For this review, use the dimensioned drawing (mm, ordinates from the lowest corner) and the shaded views. Round coordinates to 2 decimals unless told otherwise and drop trailing zeros. Order: outer loops, then holes, each group sorted by start corner. A loop starts at its lowest first (then second) coordinate and runs counter-clockwise, first axis right, second up. Notation, with made-up numbers: M 64.25,-18.5 L 89.25,-18.5 A24 cw 89.25,7.5 Z; hole C 27.25,50.5 d6. An arc over 180 degrees is marked long. Put each result on its own line as item: value.
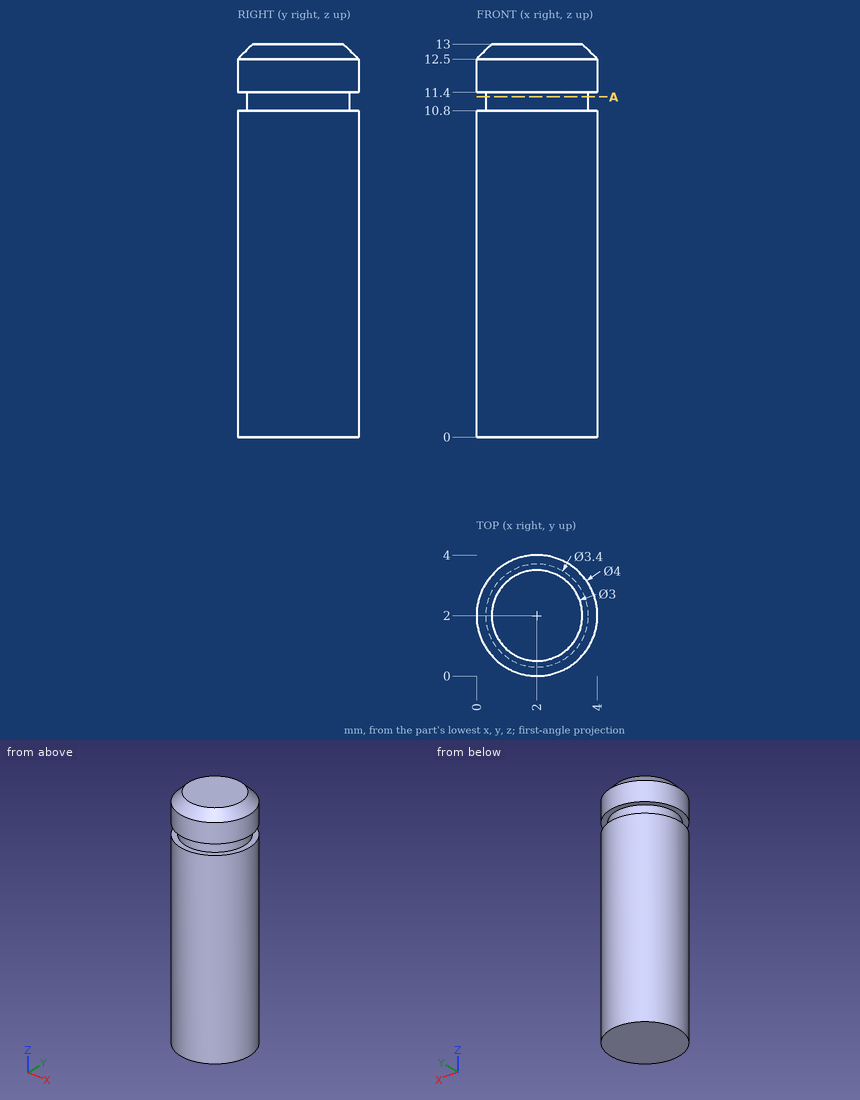
(1) To check wall thickness, follow L1, parallel to X at y = 3.05, z = 11.75; L2, parallel to Z at x = 0.25, y = 1.55; L3, parallel to Y at x = 3.55, z = 7.25. State the ranges of each line that lie inside material, in increasing order.
A:
L1: x = 0.3 to 3.7
L2: z = 0 to 10.8, 11.4 to 12.69
L3: y = 0.74 to 3.26
(2) Insertion check: pin 1 Ø1 at (x, z) = (1, 3) entering from -Y. The pin has a flat end and moves straight along its axis. Give the tip position at first contact, or say it passes through.
A:
pin 1: stops at y = 0.06
(3) Add section A-A on z = 11.25. Give the boundary of the cut face in (x, y).
A:
outline: C 2,2 d3.4
